```python
from build123d import *

# Parameters (mm, degrees)
EXTRUDE_1_DEPTH             = 5
EXTRUDE_2_DEPTH             = 5
FILLET_1_R                  = 2
CUT_EXTRUDE_1_DEPTH         = 13
FILLET_2_R                  = 2
HOLE_WIZARD_4_3_4_3_1_D     = 4.3
HOLE_WIZARD_4_3_4_3_1_DEPTH = 10.1
HOLE_WIZARD_4_3_4_3_1_TIP   = 1.291850331
SKETCH_7_W                  = 24.449376322
SKETCH_7_H                  = 27.885292322
CUT_EXTRUDE_2_DEPTH         = 10
CUT_EXTRUDE_3_DEPTH         = 10
FILLET_3_R                  = 5
SKETCH_9_W                  = 36.796643843
SKETCH_9_H                  = 32.156214513
CUT_EXTRUDE_4_DEPTH         = 21
FILLET_4_R                  = 2


with BuildPart() as part:
    # 草图1 → 凸台-拉伸1 (new body)
    with BuildSketch(Plane(origin=(0, 0, 0), x_dir=(0, 0, -1), z_dir=(1, 0, 0))):
        Polygon((-12.5, 6), (-6, 6), (-6, 61), (6, 61), (6, 6), (12.5, 6), (12.5, -6), (-12.5, -6), align=None)
    extrude(amount=EXTRUDE_1_DEPTH)

    # 草图2 → 凸台-拉伸2 (add)
    with BuildSketch(Plane.ZY):
        Polygon((-6, 61), (-12.5, 6), (12.5, 6), (6, 61), align=None)
    extrude(amount=-EXTRUDE_2_DEPTH)

    # 圆角1
    fillet_1_edges = [part.edges().sort_by_distance(p)[0] for p in [
        (2.5, 61, 6),
        (2.5, 61, -6),
    ]]
    fillet(fillet_1_edges, radius=FILLET_1_R)

    # 草图3 → 切除-拉伸1 (cut)
    with BuildSketch(Plane.ZY):
        with BuildLine():
            Line((-5.4, 2), (-5.4, -2))
            ThreePointArc((-5.4, -2), (-7.5, -4.1), (-9.6, -2))
            Line((-9.6, -2), (-9.6, 2))
            ThreePointArc((-9.6, 2), (-7.5, 4.1), (-5.4, 2))
        make_face()
        with BuildLine():
            Line((5.4, 2), (5.4, -2))
            ThreePointArc((5.4, -2), (7.5, -4.1), (9.6, -2))
            Line((9.6, -2), (9.6, 2))
            ThreePointArc((9.6, 2), (7.5, 4.1), (5.4, 2))
        make_face()
    extrude(amount=-CUT_EXTRUDE_1_DEPTH, mode=Mode.SUBTRACT)

    # 圆角2
    fillet_2_edges = [part.edges().sort_by_distance(p)[0] for p in [
        (2.5, -6, -12.5),
        (2.5, -6, 12.5),
    ]]
    fillet(fillet_2_edges, radius=FILLET_2_R)

    # Ø4.3 (4.3) 直径孔1
    with Locations(Plane.ZY):
        with Locations((0, 56), (0, 41)):
            Hole(HOLE_WIZARD_4_3_4_3_1_D / 2, depth=HOLE_WIZARD_4_3_4_3_1_DEPTH)
            with Locations((0, 0, -(HOLE_WIZARD_4_3_4_3_1_DEPTH + HOLE_WIZARD_4_3_4_3_1_TIP / 2))):  # 118° drill point
                Cone(0, HOLE_WIZARD_4_3_4_3_1_D / 2, HOLE_WIZARD_4_3_4_3_1_TIP, mode=Mode.SUBTRACT)

    # 草图7 → 切除-拉伸2 (cut)
    with BuildSketch(Plane(origin=(5, 0, 0), x_dir=(0, 0, -1), z_dir=(1, 0, 0))):
        with Locations((-1.251346032, 49.942646161)):
            Rectangle(SKETCH_7_W, SKETCH_7_H)
    extrude(amount=-CUT_EXTRUDE_2_DEPTH, mode=Mode.SUBTRACT)

    # 草图8 → 切除-拉伸3 (cut)
    with BuildSketch(Plane.ZY):
        with BuildLine():
            Line((-1, 33.75), (1, 33.75))
            ThreePointArc((1, 33.75), (3.25, 31.5), (1, 29.25))
            Line((1, 29.25), (-1, 29.25))
            ThreePointArc((-1, 29.25), (-3.25, 31.5), (-1, 33.75))
        make_face()
    extrude(amount=-CUT_EXTRUDE_3_DEPTH, mode=Mode.SUBTRACT)

    # 圆角3
    fillet_3_edges = [part.edges().sort_by_distance(p)[0] for p in [
        (2.5, 36, 8.954545455),
        (2.5, 36, -8.954545455),
    ]]
    fillet(fillet_3_edges, radius=FILLET_3_R)

    # 草图9 → 切除-拉伸4 (cut)
    with BuildSketch(Plane(origin=(5, 0, 0), x_dir=(0, 0, -1), z_dir=(1, 0, 0))):
        with Locations((-3.006475341, 22.078107257)):
            Rectangle(SKETCH_9_W, SKETCH_9_H)
    extrude(amount=-CUT_EXTRUDE_4_DEPTH, mode=Mode.SUBTRACT)

    # 圆角4
    fillet_4_edges = [part.edges().sort_by_distance(p)[0] for p in [
        (2.5, 6, 12.5),
        (2.5, 6, -12.5),
    ]]
    fillet(fillet_4_edges, radius=FILLET_4_R)


solid = part.part
```
For this review, take the finished solid that the model builds, in its own axes (mm). A direction names the side the tool comes from. Coordinates: 2 decimals unless noted, no trailing zeros. Loops run counter-clockwise (first coordinate to the right, second up) from the corner with the lowest first, then second, coordinate; pieces in that order, holes last.
1. Add section D-D, the plane y = 2.5. Give the boundary of the cut face in (x, z).
2. Add section C-C, the plane x = 0.9. Give the boundary of the cut face in (y, z), then the cut area to 3 significant figures.
3. For faces 5 (the flat face through (2, 0, 5.4)), 6 (the cylindrical face through (2.54, 5.43, 11.9)), list the 3-axis set-ups (+Z, -Z, +X, -X, +Y, -Y) from which the entire face can be reached by the end or side of a thin tool; tool diameter is ignored.
4. Add section B-B, the plane y = -1. Give the boundary of the cut face in (x, z), then the cut area to 3 significant figures.
5. Add section A-A, the plane z = -7.5. Give the boundary of the cut face in (x, y), then the cut area to 3 significant figures.
6. For line 1 (Z direction, x = 1.4, y = 0.25); line 2 (Y direction, x = 2.4, z = -7.5); line 3 (Z direction, x = 1.35, y = -3.75), list the stretches that pass through material, from the lowest coordinate up.
7. Mouldability with a two-part tool opening along Z and no side actions: class faces 1 (the cylindrical face through (2.54, -5.4, -11.93)), 2 (the cylindrical face through (2.54, -5.43, 11.9)), 3 (the flat face through (2, -6, 0)), 4 (the cylindrical face through (2.5, -4.1, 7.5)) as +Z half, -Z half, draft (parallel to the pull), parting line (faces both ways), or undercut.
Result:
1. outline: (0, -12.5) - (5, -12.5) - (5, -9.54) - (0, -9.54) - close; (0, -5.46) - (5, -5.46) - (5, 5.46) - (0, 5.46) - close; (0, 9.54) - (5, 9.54) - (5, 12.5) - (0, 12.5) - close
2. outline: (-6, -10.5) arc R2 ccw to (-4, -12.5) - (4, -12.5) arc R2 ccw to (6, -10.5) - (6, 10.5) arc R2 ccw to (4, 12.5) - (-4, 12.5) arc R2 ccw to (-6, 10.5) - close; hole (-2, -9.6) - (2, -9.6) arc R2.1 ccw to (2, -5.4) - (-2, -5.4) arc R2.1 ccw to start; hole (-2, 5.4) - (2, 5.4) arc R2.1 ccw to (2, 9.6) - (-2, 9.6) arc R2.1 ccw to start
2. area: 235 mm2
3. face 5: +X, -X
3. face 6: +Z, +X, -X, +Y
4. outline: (0, -12.5) - (5, -12.5) - (5, -9.6) - (0, -9.6) - close; (0, -5.4) - (5, -5.4) - (5, 5.4) - (0, 5.4) - close; (0, 9.6) - (5, 9.6) - (5, 12.5) - (0, 12.5) - close
4. area: 83.0 mm2
5. outline: (0, -6) - (5, -6) - (5, -4.1) - (0, -4.1) - close; (0, 4.1) - (5, 4.1) - (5, 6) - (0, 6) - close
5. area: 19.0 mm2
6. line 1: z = -12.5 to -9.6, -5.4 to 5.4, 9.6 to 12.5
6. line 2: y = -6 to -4.1, 4.1 to 6
6. line 3: z = -12.5 to -8.66, -6.34 to 6.34, 8.66 to 12.5
7. face 1: -Z half
7. face 2: +Z half
7. face 3: draft
7. face 4: undercut
